from build123d import *

# Parameters (mm, degrees)
SKETCH1_R           = 4
BOSS_EXTRUDE1_DEPTH = 50
SKETCH2_R           = 6
BOSS_EXTRUDE2_DEPTH = 6
BOSS_EXTRUDE3_DEPTH = 5
LPATTERN1_COUNT     = 2
LPATTERN1_PITCH     = 20


with BuildPart() as part:
    # Sketch1 → Boss-Extrude1 (new body)
    with BuildSketch(Plane.XY):
        Circle(SKETCH1_R)
    extrude(amount=BOSS_EXTRUDE1_DEPTH)

    # Sketch2 → Boss-Extrude2 (add)
    with BuildSketch(Plane.XY.offset(50)):
        Circle(SKETCH2_R)
    extrude(amount=BOSS_EXTRUDE2_DEPTH)

    # Sketch3 → Boss-Extrude3 (add)
    with BuildSketch(Plane(origin=(0, 0, 0), x_dir=(-1, 0, 0), z_dir=(0, 0, -1))):
        Polygon((3.321586055, 6.06931697), (-3.595389652, 5.911236389), (-6.916975707, -0.158080581), (-3.321586055, -6.06931697), (3.595389652, -5.911236389), (6.916975707, 0.158080581), align=None)
    boss_extrude3 = extrude(amount=-BOSS_EXTRUDE3_DEPTH)

    # LPattern1: Boss-Extrude3 ×2
    with Locations(*[(0, 0, i * LPATTERN1_PITCH) for i in range(1, LPATTERN1_COUNT)]):
        add(boss_extrude3)


solid = part.part
Model file for the job. Use its own axes, mm. A direction names the side the tool comes from. Round coordinates to 2 decimals unless told otherwise and drop trailing zeros. Loops run counter-clockwise (first coordinate to the right, second up) from the corner with the lowest first, then second, coordinate; pieces in that order, holes last.
1. Band-saw the part on A-A, the plane y = -4.5. List the corners of the cut face in (x, z), and give its area (3 significant figures).
Check values:
outline: (-4.37, 0) - (4.28, 0) - (4.28, 5) - (-4.37, 5) - close; (-4.37, 20) - (4.28, 20) - (4.28, 25) - (-4.37, 25) - close; (-3.97, 50) - (3.97, 50) - (3.97, 56) - (-3.97, 56) - close
area: 134 mm2
2. Band-saw the part on C-C, the plane z = 4.5. List the corners of the cut face in (x, y).
Check values:
outline: (-6.92, 0.16) - (-3.6, -5.91) - (3.32, -6.07) - (6.92, -0.16) - (3.6, 5.91) - (-3.32, 6.07) - close
3. Mould opens along Z. For faces 1 (the cylindrical face through (-0.867, -3.905, 12.395)), 2 (the flat face through (-5.144, 3.072, 2.465)), 3 (the flat face through (0, 0, 56)) say: +Z half, -Z half, draft (parallel to the pull), parting line (faces both ways), or undercut.
Check values:
face 1: undercut
face 2: draft
face 3: +Z half
4. Tool access for faces 4 (the flat face through (0, 0, 0)), 5 (the flat face through (-3, 3, 25)), 6 (the cylindrical face through (-6, 0, 53)): list every direction of +Z, -Z, +X, -X, +Y, -Y with a clear straight run to the whole face (end or side of a thin tool).
Check values:
face 4: -Z, +X, -X, +Y, -Y
face 5: none
face 6: +Z
5. Band-saw the part on D-D, the plane x = -0.5. List the corners of the cut face in (y, z), and give its area (3 significant figures).
Check values:
outline: (-5.98, 0) - (6, 0) - (6, 5) - (3.97, 5) - (3.97, 20) - (6, 20) - (6, 25) - (3.97, 25) - (3.97, 50) - (5.98, 50) - (5.98, 56) - (-5.98, 56) - (-5.98, 50) - (-3.97, 50) - (-3.97, 25) - (-5.98, 25) - (-5.98, 20) - (-3.97, 20) - (-3.97, 5) - (-5.98, 5) - close
area: 509 mm2
6. Drop flat-ended pins along their axis: P1, Ø1.5, axis at y = 2.5, z = 9, coming from the +X side; P2, Ø3, axis at y = 4, z = 46, coming from the +X side; P3, Ø6, axis at x = 1.5, y = 3, coming from the -Z side; P4, Ø1.5, axis at y = 1.5, z = 49, coming from the +X side. Give the stop position or say it passes through.
Check values:
P1: stops at x = 3.6
P2: stops at x = 3.12
P3: stops at z = 0
P4: stops at x = 3.93
7. Band-saw the part on B-B, the plane x = 5. List the corners of the cut face in (y, z), and give its area (3 significant figures).
Check values:
outline: (-3.32, 50) - (3.32, 50) - (3.32, 56) - (-3.32, 56) - close; (-3.31, 0) - (3.34, 0) - (3.34, 5) - (-3.31, 5) - close; (-3.31, 20) - (3.34, 20) - (3.34, 25) - (-3.31, 25) - close
area: 106 mm2
8. Wall check: probe 1 along Z at (x, y) = (-2.75, 3.25); probe 2 along Y at (x, z) = (0, 8); probe 3 along Y at (x, z) = (3.25, 53.5). Give the ranges that are in metal, low to high.
Check values:
probe 1: z = 0 to 5, 20 to 25, 50 to 56
probe 2: y = -4 to 4
probe 3: y = -5.04 to 5.04
